Drawing for the job (mm, zero at the part's lowest x, y, z). A direction names the side the tool comes from. Give positions to 0.01 mm unless a question says otherwise; leave off trailing zeros. Loops run counter-clockwise (first coordinate to the right, second up) from the corner with the lowest first, then second, coordinate; pieces in that order, holes last. Notation, with made-up numbers: (-21.75, -29) -> (23.25, -29) arc R19 ccw to (23.25, -10) -> close; hole circle Ø3 at (48.5, -8). An arc over 180 degrees is marked (long way). Answer in a Markdown table with one row per item. Add a question column.
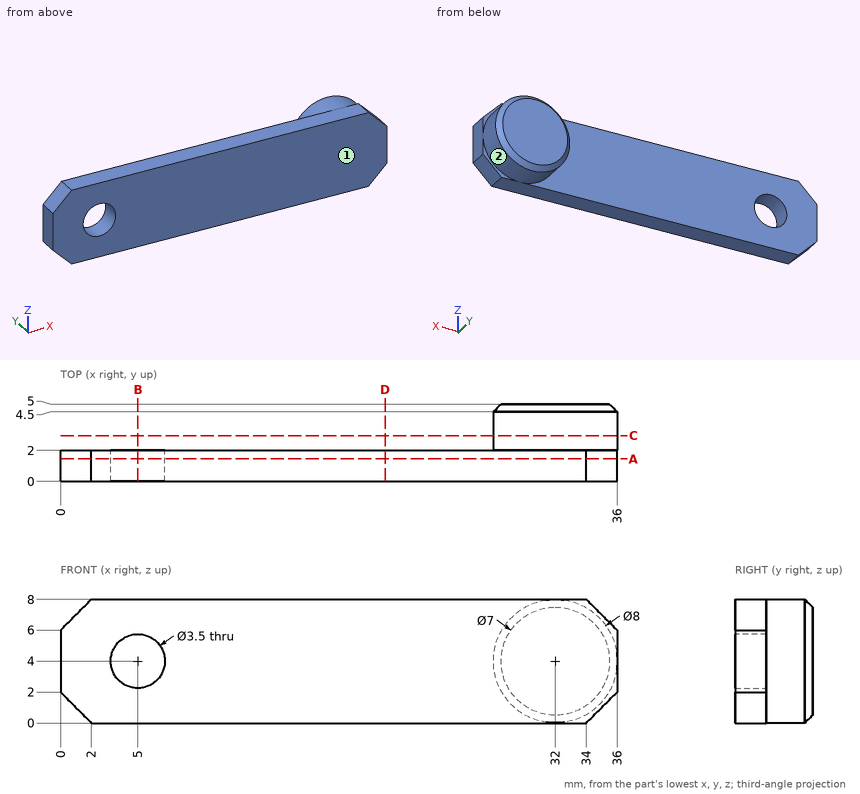
(1) 3-axis set-ups, long thin cutter, end or side, ignore diameter. For the marked faces 1 and 2: which of +Z, -Z, +X, -X, +Y, -Y reach the whole face in a straight line?
(2) Saw through at B-B, the plane x = 5. List the corners of the cut face in (y, z).
(3) Saw through at A-A, the plane y = 1.45. List the corners of the cut face in (x, z), then the cut area to 3 significant figures.
(4) Wall check: line 1 along X through (y, z) = (0.5, 4); line 2 along Y through (x, z) = (25, 7); line 3 along Z through (x, y) = (34.5, 1.5). Give the ranges that are in metal, low to high. Write a range as from..to.
(5) Saw through at D-D, the plane x = 21. List the corners of the cut face in (y, z), then the cut area to 3 significant figures.
(6) Flat gauge pins, fed straight in: pin 1 Ø1 at (x, y) = (8, 3) entering from +Z; pin 2 Ø3 at (x, z) = (19, 1.5) entering from +Y. Where does each tip first touch, or does it go through?
(7) Saw through at C-C, the plane y = 2.95. List the corners of the cut face in (x, z), then the cut area to 3 significant figures.
Worked answers:
| question | item | result |
|---|---|---|
| 1 | face 1 | +Z, -Z, +X, -X, -Y |
| 1 | face 2 | +Y |
| 2 | outline | (0, 0) -> (2, 0) -> (2, 2.25) -> (0, 2.25) -> close; (0, 5.75) -> (2, 5.75) -> (2, 8) -> (0, 8) -> close |
| 3 | outline | (0, 2) -> (2, 0) -> (34, 0) -> (36, 2) -> (36, 6) -> (34, 8) -> (2, 8) -> (0, 6) -> close; hole circle Ø3.5 at (5, 4) |
| 3 | area | 270 mm^2 |
| 4 | line 1 | 0..3.25, 6.75..36 |
| 4 | line 2 | 0..2 |
| 4 | line 3 | 0.5..7.5 |
| 5 | outline | (0, 0) -> (2, 0) -> (2, 8) -> (0, 8) -> close |
| 5 | area | 16.0 mm^2 |
| 6 | pin 1 | through |
| 6 | pin 2 | y = 2 |
| 7 | outline | circle Ø8 at (32, 4) |
| 7 | area | 50.3 mm^2 |
